Geometry check sheet. Reference: the model listing, model coordinates, mm. Face numbers are marked on the shaded views. A direction names the side the tool comes from. Coordinates: 2 decimals unless noted, no trailing zeros. Write each loop counter-clockwise with the first axis right and the second up, starting at its lowest first coordinate (ties: lowest second). Pieces come first, ordered by that corner, then holes. Notation, with made-up numbers: M 21.25,-22 L 38.25,-22 A18 ccw 38.25,-11 Z; hole C -4.5,-1 d6. An arc over 180 degrees is marked long. Write each question's results on one line, items separated by ' | '.
```python
from build123d import *

# Parameters (mm, degrees)
BASE_BLOCK_SKETCH_W           = 90
BASE_BLOCK_SKETCH_H           = 48
BASE_BLOCK_DEPTH              = 12
CRADLE_CUT_DEPTH              = 40
CLAMP_BOSS_SKETCH_R           = 28
CLAMP_BOSS_SKETCH_R_2         = 16
CLAMP_BOSS_56_DEPTH           = 56
BORE_AND_SPLIT_SLOT_CUT_DEPTH = 56


with BuildPart() as part:
    # Base Block Sketch → Base Block (new, symmetric)
    with BuildSketch(Plane.XY):
        Rectangle(BASE_BLOCK_SKETCH_W, BASE_BLOCK_SKETCH_H)
    extrude(amount=BASE_BLOCK_DEPTH, both=True)

    # Cradle Cut Sketch → Cradle Cut (cut)
    with BuildSketch(Plane.ZY.offset(45)):
        with BuildLine():
            Line((12, -16), (12, 16))
            ThreePointArc((12, 16), (-4, 0), (12, -16))
        make_face()
    extrude(amount=-CRADLE_CUT_DEPTH, mode=Mode.SUBTRACT)

    # Clamp Boss Sketch → Clamp Boss Ø56 (add)
    with BuildSketch(Plane(origin=(0, 0, -12), x_dir=(-1, 0, 0), z_dir=(0, 0, -1))):
        with Locations((-45, 0)):
            Circle(CLAMP_BOSS_SKETCH_R)
        with Locations((-45, 0)):
            Circle(CLAMP_BOSS_SKETCH_R_2, mode=Mode.SUBTRACT)
    extrude(amount=-CLAMP_BOSS_56_DEPTH)

    # Bore and Split Slot Sketch → Bore and Split Slot Cut (cut)
    with BuildSketch(Plane.XY.offset(44)):
        Polygon((57.677488521, -2.241298623), (57.677488521, 0.758701377), (76.626798925, 0.758701377), (76.626798925, -5.241298623), (57.677488521, -5.241298623), align=None)
    extrude(amount=-BORE_AND_SPLIT_SLOT_CUT_DEPTH, mode=Mode.SUBTRACT)


solid = part.part
```
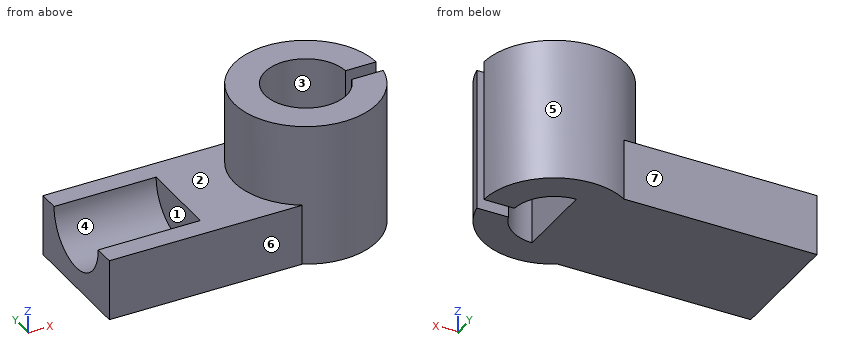
Q1. Sectioned sample at C-C on x = 25. Record the cut outline in (y, z), and give its area (3 significant figures).
Geometry check:
outline: M -24,-12 L 24,-12 L 24,12 L 19.6,12 L 19.6,44 L -19.6,44 L -19.6,12 L -24,12 Z | area: 2,410 mm2
Q2. Depth check by flat-ended pin: P1, Ø13, axis at x = 38.5, y = 0.5, coming from the +Z side; P2, Ø6, axis at y = -22, z = 18, coming from the +X side; P3, Ø2, axis at x = -19.5, y = -7, coming from the +Z side. Enter the tip coordinate at first touch or a pass-through.
Geometry check:
P1: stops at z = 12 | P2: stops at x = 65.57 | P3: stops at z = -1.86
Q3. Sectioned sample at A-A on x = 48.5. Record the cut outline in (y, z), and give its area (3 significant figures).
Geometry check:
outline: M -27.78,-12 L -15.61,-12 L -15.61,44 L -27.78,44 Z; M 15.61,-12 L 27.78,-12 L 27.78,44 L 15.61,44 Z | area: 1,360 mm2
Q4. Sectioned sample at B-B on y = 10. Record the cut outline in (x, z), and give its area (3 significant figures).
Geometry check:
outline: M -45,-12 L 45,-12 L 45,12 L 32.51,12 L 32.51,44 L 18.85,44 L 18.85,12 L -5,12 L -5,-0.49 L -45,-0.49 Z; M 57.49,-12 L 71.15,-12 L 71.15,44 L 57.49,44 Z | area: 2,860 mm2
Q5. Mould release check, pull along X, two halves, no side actions. Record for the marked faces 1, 2 and 3: pulls with the +X half, pulls with the -X half, needs draft (parallel to the pull), parting line crosses it, or undercut.
Geometry check:
face 1: pulls with the -X half | face 2: needs draft | face 3: undercut
Q6. Sectioned sample at D-D on y = 18.5. Record the cut outline in (x, z).
Geometry check:
outline: M -45,-12 L 66.02,-12 L 66.02,44 L 23.98,44 L 23.98,12 L -45,12 Z
Q7. Scan lines: probe 1 along Y at (x, z) = (45, 16); probe 2 along X at (y, z) = (0, 0.5); probe 3 along Y at (x, z) = (52.5, 12.5). Record each from-to range of solid material in increasing order.
Geometry check:
probe 1: y = -28 to -16, 16 to 28 | probe 2: x = -5 to 45 | probe 3: y = -26.98 to -14.13, 14.13 to 26.98
Q8. Access from +Z, -Z, +X, -X, +Y, -Y to the whole of each face (thin tool, end or side, straight path). Record for the marked faces 4, 5, 6 and 7.
Geometry check:
face 4: +Z, -X | face 5: +Z | face 6: +Z, -Z, -X, -Y | face 7: +Z, -Z, -X, +Y
